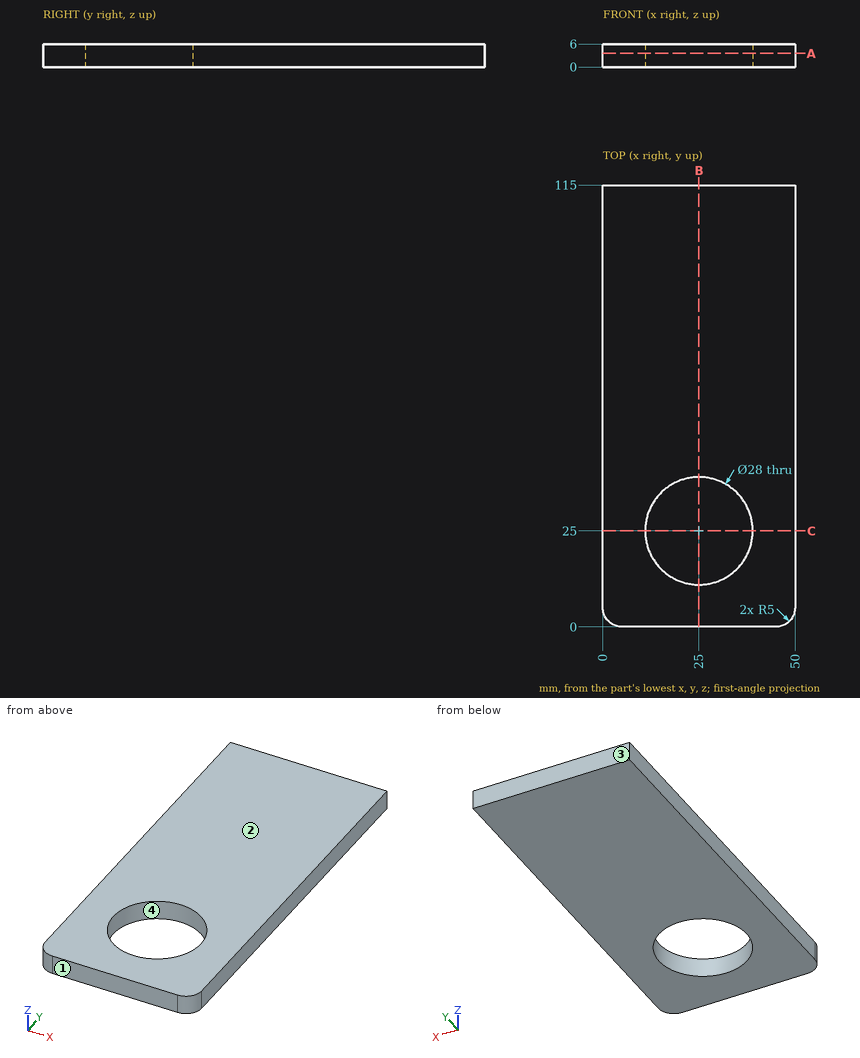
Answer from the drawing. Dimensions are ordinates in mm from the lowest x, y and z of the part. Give positions to 0.01 mm unless a question says otherwise; leave off trailing zeros. Loops run counter-clockwise (first coordinate to the right, second up) from the corner with the lowest first, then second, coordinate; pieces in that order, holes last. Notation, with made-up numbers: (65.25, -2) - (72.25, -2) arc R15 cw to (72.25, 14) - close; hole circle Ø9 at (82.5, 32.5). An arc over 180 degrees is marked (long way). Answer as a JSON object with one key per item and string values.
1. For a pull along Y with two mould halves and no side action, classify the marked faces 1, 2, 3 and 4 as pulls with the +Y half, pulls with the -Y half, needs draft (parallel to the pull), parting line crosses it, or undercut.
Determined:
{"face 1": "pulls with the -Y half", "face 2": "needs draft", "face 3": "pulls with the +Y half", "face 4": "undercut"}
2. A cutting plane is placed at B-B (x = 25). Write down the section's boundary in (y, z), then the cut area to 3 significant figures.
Determined:
{"outline": "(0, 0) - (11, 0) - (11, 6) - (0, 6) - close; (39, 0) - (115, 0) - (115, 6) - (39, 6) - close", "area": "522 mm²"}
3. A cutting plane is placed at C-C (y = 25). Write down the section's boundary in (x, z), then the cut area to 3 significant figures.
Determined:
{"outline": "(0, 0) - (11, 0) - (11, 6) - (0, 6) - close; (39, 0) - (50, 0) - (50, 6) - (39, 6) - close", "area": "132 mm²"}
4. A cutting plane is placed at A-A (z = 3.55). Write down the section's boundary in (x, y).
Determined:
{"outline": "(0, 5) arc R5 ccw to (5, 0) - (45, 0) arc R5 ccw to (50, 5) - (50, 115) - (0, 115) - close; hole circle Ø28 at (25, 25)"}
5. Find the intervals of material crossed by L1, parallel to Y at x = 25, z = 4.25; L2, parallel to Y at x = 12.5, z = 1.6; L3, parallel to Y at x = 46.5, z = 1.8, in increasing order. Write a range as [from, to].
Determined:
{"L1": "[0, 11], [39, 115]", "L2": "[0, 18.7], [31.3, 115]", "L3": "[0.23, 115]"}
